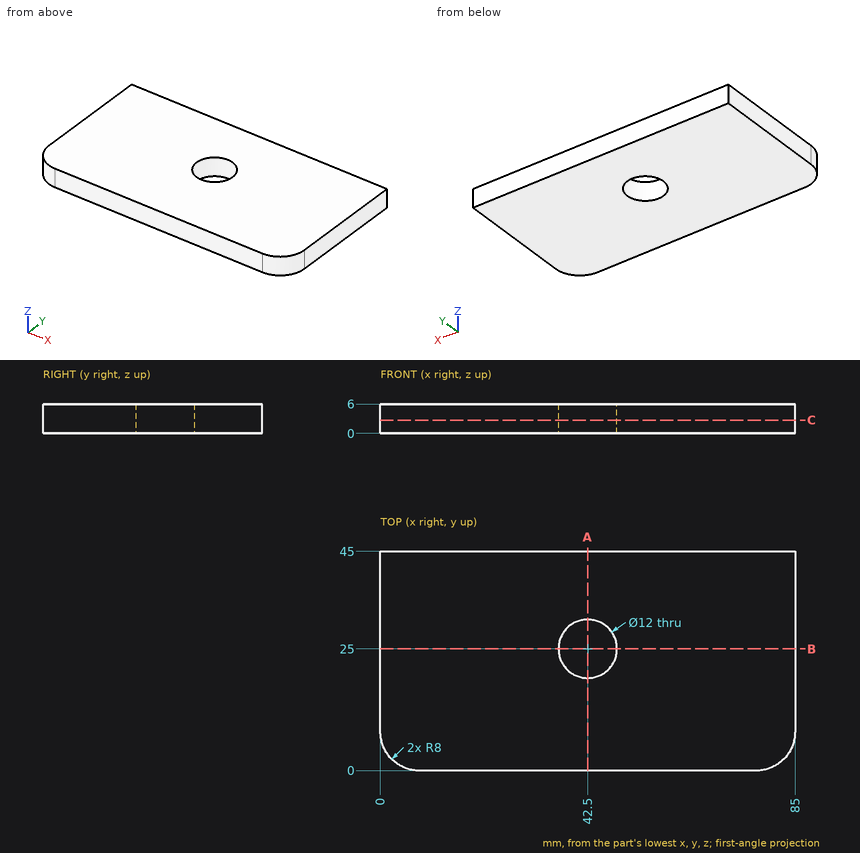
Here's the drawing with two shaded views (mm, measured from the low corner). I have some questions. Coordinates: 2 decimals unless noted, no trailing zeros. Write each loop counter-clockwise with the first axis right and the second up, starting at its lowest first coordinate (ties: lowest second). Pieces come first, ordered by that corner, then holes. Notation, with made-up numbers: (68, -19) -> (73, -19) arc R16 cw to (73, 10) -> close; hole circle Ø7 at (48.5, 70.25). An arc over 180 degrees is marked (long way). Use a Markdown table: item, result. Add a question column.
(1) If we section it at C-C, the plane z = 2.7: Write out the boundary of the cut face in (x, y), and give its area (3 significant figures).
(2) Please list where these lines run through material, in increasing order: line 1 (Y direction, x = 42.5, z = 3.1); line 2 (X direction, y = 23.5, z = 2.9); line 3 (X direction, y = 25.5, z = 1.2).
(3) If we section it at B-B, the plane y = 25: Write out the boundary of the cut face in (x, z).
(4) If we section it at A-A, the plane x = 42.5: Write out the boundary of the cut face in (y, z), and give its area (3 significant figures).
Outcome:
| question | item | result |
|---|---|---|
| 1 | outline | (0, 8) arc R8 ccw to (8, 0) -> (77, 0) arc R8 ccw to (85, 8) -> (85, 45) -> (0, 45) -> close; hole circle Ø12 at (42.5, 25) |
| 1 | area | 3,680 mm^2 |
| 2 | line 1 | y = 0 to 19, 31 to 45 |
| 2 | line 2 | x = 0 to 36.69, 48.31 to 85 |
| 2 | line 3 | x = 0 to 36.52, 48.48 to 85 |
| 3 | outline | (0, 0) -> (36.5, 0) -> (36.5, 6) -> (0, 6) -> close; (48.5, 0) -> (85, 0) -> (85, 6) -> (48.5, 6) -> close |
| 4 | outline | (0, 0) -> (19, 0) -> (19, 6) -> (0, 6) -> close; (31, 0) -> (45, 0) -> (45, 6) -> (31, 6) -> close |
| 4 | area | 198 mm^2 |
